```python
from build123d import *

# Parameters (mm, degrees)
SKETCH1_W           = 381
SKETCH1_H           = 230
BOSS_EXTRUDE1_DEPTH = 5
F_15_HOLE1_D        = 15
FILLET2_R           = 5


with BuildPart() as part:
    # Sketch1 → Boss-Extrude1 (new, symmetric)
    with BuildSketch(Plane.XY):
        Rectangle(SKETCH1_W, SKETCH1_H)
    extrude(amount=BOSS_EXTRUDE1_DEPTH, both=True)

    # Ø15 Hole1 (through all)
    with Locations(Plane.XY.offset(5)):
        with Locations((-167.5, 95), (167.5, 95), (167.5, -95), (-167.5, -95)):
            Hole(F_15_HOLE1_D / 2)

    # Fillet2
    fillet2_edges = [part.edges().sort_by_distance(p)[0] for p in [
        (-190.5, 115, 0),
        (190.5, 115, 0),
        (190.5, -115, 0),
        (-190.5, -115, 0),
    ]]
    fillet(fillet2_edges, radius=FILLET2_R)


solid = part.part
```
For this review, take the finished solid that the model builds, in its own axes (mm). Coordinates: 2 decimals unless noted, no trailing zeros. Order: outer loops, then holes, each group sorted by start corner. A loop starts at its lowest first (then second) coordinate and runs counter-clockwise, first axis right, second up. Notation, with made-up numbers: (2.5, 0.5) -> (58.5, 0.5) arc R26 ccw to (58.5, 28.5) -> close; hole circle Ø10 at (23.5, 24). An arc over 180 degrees is marked (long way). Use CSV: the item, a comma, the result in double quotes. Start each with the question number.
Item 1: We need section B-B, the plane x = 167.5. Give the boundary of the cut face in (y, z).
Item 2: Draft analysis for pull direction X (two halves, no side actions). For faces 1 (the face through (190.5, -2, 0)), 2 (the face through (-3, 2, -5)), 3 (the face through (-174.43, -97.87, -0.07)), state which applies: pulls with the +X half, pulls with the -X half, needs draft (parallel to the pull), parting line crosses it, or undercut.
Item 3: Insertion check: pin 1 (9 mm diameter, centred on x = -167.5, y = -95, fed in from +Z); pin 2 (17 mm diameter, centred on x = 167.5, y = -95, fed in from +Z). Each pin has a flat end and moves straight along its axis. Give the tip position at first contact, or say it passes through.
Item 4: We need section A-A, the plane y = -95. Give the boundary of the cut face in (x, z).
Item 5: Wall thickness on probe 1 along Y at (x, z) = (-167.5, 3.5); probe 2 along X at (y, z) = (101, -1.75): over which ranges is each line inside the solid? List them lowest first.
Derived:
1,outline,"(-115, -5) -> (-102.5, -5) -> (-102.5, 5) -> (-115, 5) -> close; (-87.5, -5) -> (87.5, -5) -> (87.5, 5) -> (-87.5, 5) -> close; (102.5, -5) -> (115, -5) -> (115, 5) -> (102.5, 5) -> close"
2,face 1,"pulls with the +X half"
2,face 2,"needs draft"
2,face 3,"undercut"
3,pin 1,"passes through"
3,pin 2,"stops at z = 5"
4,outline,"(-190.5, -5) -> (-175, -5) -> (-175, 5) -> (-190.5, 5) -> close; (-160, -5) -> (160, -5) -> (160, 5) -> (-160, 5) -> close; (175, -5) -> (190.5, -5) -> (190.5, 5) -> (175, 5) -> close"
5,probe 1,"y = -115 to -102.5, -87.5 to 87.5, 102.5 to 115"
5,probe 2,"x = -190.5 to -172, -163 to 163, 172 to 190.5"
